from build123d import *

# Parameters (mm, degrees)
EXTRUDE_390_DEPTH = 4
FILLET_1290_R     = 0.25


with BuildPart() as part:
    # 草图1 → Extrude 390 (new body)
    with BuildSketch(Plane(origin=(0, 0, 0), x_dir=(0, 0, -1), z_dir=(1, 0, 0))):
        Polygon((5, 2.886751346), (5, -2.886751346), (0, -5.773502692), (-5, -2.886751346), (-5, 2.886751346), (0, 5.773502692), align=None)
    extrude(amount=EXTRUDE_390_DEPTH)

    # 草图2 → 凸台-旋转1 (revolve)
    with BuildSketch(Plane.XY, mode=Mode.PRIVATE) as revolve_1_sk:
        Polygon((0, 0), (44, 0), (44, 2.134), (44, 3), (0, 3), align=None)
    revolve(revolve_1_sk.sketch.rotate(Axis((0, 0, 0), (1, 0, 0)), 90), axis=Axis((0, 0, 0), (1, 0, 0)))

    # 草图3 → 切除-旋转1 (revolve, cut)
    with BuildSketch(Plane.XY):
        Polygon((0, 5), (3.333333333, 10.773502692), (3.333333333, 15.773502692), (-10, 15.773502692), (-10, 5), align=None)
    revolve(axis=Axis((0, 0, 0), (1, 0, 0)), mode=Mode.SUBTRACT)

    # 草图4 → 切除-旋转3 (revolve, cut)
    with BuildSketch(Plane.XY, mode=Mode.PRIVATE) as cut_revolve_3_sk:
        Polygon((4, 4.44), (3.5, 4.728675135), (3.5, 5.773502692), (4, 5.773502692), align=None)
    revolve(cut_revolve_3_sk.sketch.rotate(Axis((0, 0, 0), (1, 0, 0)), 90), axis=Axis((0, 0, 0), (1, 0, 0)), mode=Mode.SUBTRACT)

    # Fillet 1290
    fillet_1290_edges = [part.edges().sort_by_distance(p)[0] for p in [
        (4, 0, -3),
    ]]
    fillet(fillet_1290_edges, radius=FILLET_1290_R)

    # 草图6 → 切除-旋转4 (revolve, cut)
    with BuildSketch(Plane.XY, mode=Mode.PRIVATE) as cut_revolve_4_sk:
        Polygon((43.5, 3), (44.5, 3), (44, 2.133974596), align=None)
    revolve(cut_revolve_4_sk.sketch.rotate(Axis((0, 0, 0), (1, 0, 0)), 90), axis=Axis((0, 0, 0), (1, 0, 0)), mode=Mode.SUBTRACT)


solid = part.part
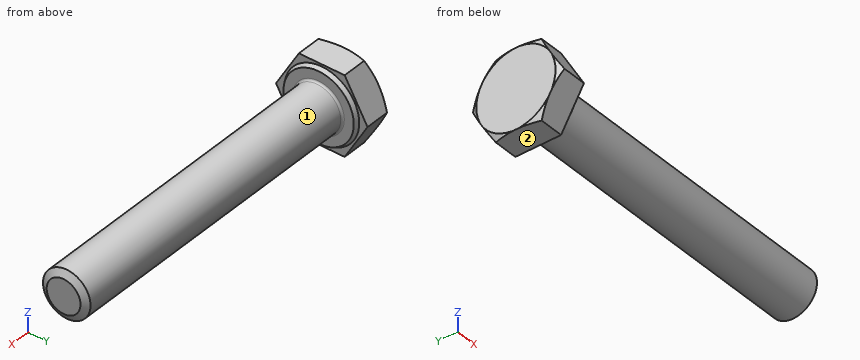
Build history of the part. All positions in model axes, mm. Face numbers are marked on the shaded views. A direction names the side the tool comes from. Round coordinates to 2 decimals unless told otherwise and drop trailing zeros. Loops run counter-clockwise (first coordinate to the right, second up) from the corner with the lowest first, then second, coordinate; pieces in that order, holes last. Notation, with made-up numbers: (44, 78) -> (57, 78) arc R29 cw to (57, 104) -> close; hole circle Ø1 at (56, 13.25). An arc over 180 degrees is marked (long way). Answer in a Markdown table with one row per item.
Item 1: Which spindle directions (+Z, -Z, +X, -X, +Y, -Y) get a long thin tool onto all of the face, cutting with end or side? Do the marked faces 1 and 2. Say none if no direction does.
Answers below:
| item | result |
|---|---|
| face 1 | +X |
| face 2 | -Z, +X, -X, +Y, -Y |
Item 2: Saw through at A-A (x = 7). Write the cut outline in (y, z), and give its area (3 significant figures).
Answers below:
| item | result |
|---|---|
| outline | circle Ø6 at (0, 0) |
| area | 28.3 mm² |
Item 3: Pin check, flat tips, straight feed: pin 1 (3 mm diameter, centred on x = 13.5, y = 1, fed in from +Z); pin 2 (4 mm diameter, centred on x = 20.5, y = -1.5, fed in from -Z); pin 3 (3 mm diameter, centred on y = -2.5, z = -0.5, fed in from +X); pin 4 (6 mm diameter, centred on x = 20.5, z = -3, fed in from -Y). Stop position of each tip, or through.
Answers below:
| item | result |
|---|---|
| pin 1 | stops at z = 3 |
| pin 2 | stops at z = -3 |
| pin 3 | stops at x = 44 |
| pin 4 | stops at y = -3 |
Item 4: Drill centre lines: L1, parallel to X at y = -4.75, z = 1; L2, parallel to X at y = -2, z = -3; L3, parallel to Y at x = 2, z = 2.5. Where is each one in solid material? Low to high. Write a range as [from, to].
Answers below:
| item | result |
|---|---|
| L1 | x = [0, 3.5] |
| L2 | x = [0, 4] |
| L3 | y = [-4.33, 4.33] |
